Part model, mm, in its own coordinate system. Face numbers are marked on the shaded views. A direction names the side the tool comes from. Give positions to 0.01 mm unless a question says otherwise; leave off trailing zeros. Order: outer loops, then holes, each group sorted by start corner. A loop starts at its lowest first (then second) coordinate and runs counter-clockwise, first axis right, second up.
1. Slice it at D-D on x = -17. List the corners of the cut face in (y, z).
2. Which spindle directions (+Z, -Z, +X, -X, +Y, -Y) get a long thin tool onto all of the face, cutting with end or side? Do the marked faces 1, 2 and 3. Say none if no direction does.
3. Probe line 1 (Y direction, x = 0, z = 14.15); line 2 (Y direction, x = -6, z = 3.5); line 3 (Y direction, x = -6.5, z = 14.25). List the from-to ranges inside material, lowest first.
4. Slice it at A-A on x = 0. List the corners of the cut face in (y, z), and give its area (3 significant figures).
5. Slice it at C-C on x = -7. List the corners of the cut face in (y, z).
6. Drop flat-ended pins along their axis: pin 1 Ø5 at (x, y) = (2.5, 28) entering from +Z; pin 2 Ø3.5 at (y, z) = (21, 5.5) entering from +X; pin 3 Ø3 at (x, z) = (15.5, 12.5) entering from +Y. Give the stop position or say it passes through.
7. Slice it at B-B on z = 14.5. List the corners of the cut face in (x, y), and give its area (3 significant figures).
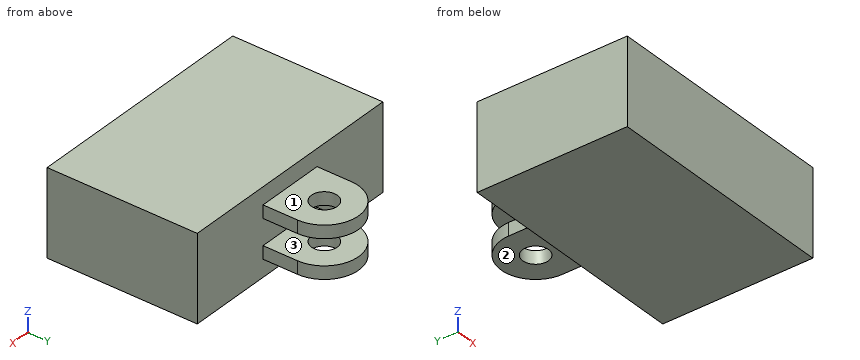
from build123d import *

# Parameters (mm, degrees)
SKETCH1_W               = 55
SKETCH1_H               = 35
BOSS_EXTRUDE1_DEPTH     = 20
SKETCH2_W               = 16
SKETCH2_H               = 12
BOSS_EXTRUDE2_DEPTH     = 16
CUT_EXTRUDE1_DEPTH      = 62.296410988
CUT_EXTRUDE1_DEPTH_BACK = 16
SKETCH3_W               = 16
SKETCH3_H               = 6
SKETCH4_R               = 3
CUT_EXTRUDE2_DEPTH      = 47.200649346


with BuildPart() as part:
    # Sketch1 → Boss-Extrude1 (new body)
    with BuildSketch(Plane.XY):
        Rectangle(SKETCH1_W, SKETCH1_H)
    extrude(amount=BOSS_EXTRUDE1_DEPTH)

    # Sketch2 → Boss-Extrude2 (add)
    with BuildSketch(Plane(origin=(0, 17.5, 0), x_dir=(1, 0, 0), z_dir=(0, 1, 0))):
        with Locations((0, -10)):
            Rectangle(SKETCH2_W, SKETCH2_H)
    extrude(amount=BOSS_EXTRUDE2_DEPTH)

    # Sketch3 → Cut-Extrude1 (cut, two sides: drawn at the far end of the back side and taken through both)
    with BuildSketch(Plane(origin=(0, 33.5, 0), x_dir=(1, 0, 0), z_dir=(0, 1, 0)).offset(-CUT_EXTRUDE1_DEPTH_BACK)):
        with Locations((0, -10)):
            Rectangle(SKETCH3_W, SKETCH3_H)
    extrude(amount=CUT_EXTRUDE1_DEPTH + CUT_EXTRUDE1_DEPTH_BACK, mode=Mode.SUBTRACT)

    # Sketch4 → Cut-Extrude2 (cut, through all)
    with BuildSketch(Plane.XY.offset(16)):
        with Locations((0, 25.5)):
            Circle(SKETCH4_R)
        with BuildLine():
            Line((-8, 25.5), (-21.64466881, 27.690296909))
            Line((-21.64466881, 27.690296909), (-8, 39.036178495))
            Line((-8, 39.036178495), (25.748849804, 31.989915092))
            Line((25.748849804, 31.989915092), (8, 25.5))
            ThreePointArc((8, 25.5), (0, 33.5), (-8, 25.5))
        make_face()
    extrude(amount=-CUT_EXTRUDE2_DEPTH, mode=Mode.SUBTRACT)


solid = part.part
Data:
1. outline: (-17.5, 0) - (17.5, 0) - (17.5, 20) - (-17.5, 20) - close
2. face 1: +Z, +X, -X, +Y
2. face 2: -Z, +X, -X, +Y
2. face 3: +X, -X, +Y
3. line 1: y = -17.5 to 22.5, 28.5 to 33.5
3. line 2: y = -17.5 to 17.5
3. line 3: y = -17.5 to 30.16
4. outline: (-17.5, 0) - (17.5, 0) - (17.5, 4) - (22.5, 4) - (22.5, 7) - (17.5, 7) - (17.5, 13) - (22.5, 13) - (22.5, 16) - (17.5, 16) - (17.5, 20) - (-17.5, 20) - close; (28.5, 4) - (33.5, 4) - (33.5, 7) - (28.5, 7) - close; (28.5, 13) - (33.5, 13) - (33.5, 16) - (28.5, 16) - close
4. area: 760 mm2
5. outline: (-17.5, 0) - (17.5, 0) - (17.5, 4) - (29.37, 4) - (29.37, 7) - (17.5, 7) - (17.5, 13) - (29.37, 13) - (29.37, 16) - (17.5, 16) - (17.5, 20) - (-17.5, 20) - close
6. pin 1: stops at z = 16
6. pin 2: stops at x = 8
6. pin 3: stops at y = 17.5
7. outline: (-27.5, -17.5) - (27.5, -17.5) - (27.5, 17.5) - (8, 17.5) - (8, 25.5) arc R8 ccw to (-8, 25.5) - (-8, 17.5) - (-27.5, 17.5) - close; hole circle Ø6 at (0, 25.5)
7. area: 2,130 mm2
